The listing builds one solid part. Answer for the finished solid, in the listing's coordinates (mm). Coordinates: 2 decimals unless noted, no trailing zeros. Loops run counter-clockwise (first coordinate to the right, second up) from the corner with the lowest first, then second, coordinate; pieces in that order, holes last. Notation, with made-up numbers: M 40,71.25 L 93,71.25 A13 cw 93,95.25 Z; hole C 7,-29 d3. An arc over 180 degrees is marked long. Return JSON: item names as keys, results as strings. Group by question number.
1. Section A-A (z = -1.5) is taken. Write down the section's boundary in (x, y), then the cut area to 3 significant figures.
2. Section B-B (y = -175) is taken. Write down the section's boundary in (x, z).
3. Straight lines are drawn through the part: L1, parallel to Y at x = 4, z = -1.4; L2, parallel to Y at x = 3.25, z = 2.5; L3, parallel to X at y = -223.5, z = 0.25. For each, find the intervals that lie inside material, in ascending order. Write a range as from..to.
```python
from build123d import *

# Parameters (mm, degrees)
BOSS_EXTRUDE1_DEPTH = 400
CUT_EXTRUDE1_DEPTH  = 401.196201881
SKETCH3_R           = 1.75
CUT_EXTRUDE2_DEPTH  = 401.196201985


with BuildPart() as part:
    # Sketch1 → Boss-Extrude1 (new body)
    with BuildSketch(Plane(origin=(0, 0, 0), x_dir=(1, 0, 0), z_dir=(0, 1, 0))):
        with BuildLine():
            Line((0, 3), (8, 3))
            ThreePointArc((8, 3), (11, 0), (8, -3))
            Line((8, -3), (0, -3))
            ThreePointArc((0, -3), (-3, 0), (0, 3))
        make_face()
    extrude(amount=-BOSS_EXTRUDE1_DEPTH)

    # Sketch2 → Cut-Extrude1 (cut, through all)
    with BuildSketch(Plane(origin=(0, 0, -3), x_dir=(-1, 0, 0), z_dir=(0, 0, -1))):
        with BuildLine():
            Line((9.595782006, 3.055219164), (9.595782006, -10.123279697))
            Line((9.595782006, -10.123279697), (3.026265269, -10.123279697))
            ThreePointArc((3.026265269, -10.123279697), (-4, 0), (-11.026265269, -10.123279697))
            Line((-11.026265269, -10.123279697), (-18.139014199, -10.123279697))
            Line((-18.139014199, -10.123279697), (-18.139014199, 3.055219164))
            Line((-18.139014199, 3.055219164), (9.595782006, 3.055219164))
        make_face()
    extrude(amount=-CUT_EXTRUDE1_DEPTH, mode=Mode.SUBTRACT)

    # Sketch3 → Cut-Extrude2 (cut, through all)
    with BuildSketch(Plane.XY.offset(3)):
        with Locations((4, -7.883965637)):
            Circle(SKETCH3_R)
    extrude(amount=-CUT_EXTRUDE2_DEPTH, mode=Mode.SUBTRACT)


solid = part.part
```
Worked out:
{
 "1": {"outline": "M -2.6,-400 L 10.6,-400 L 10.6,-3.93 A7.5 ccw -2.6,-3.93 Z; hole C 4,-7.88 d3.5", "area": "5,250 mm^2"},
 "2": {"outline": "M 0,-3 L 8,-3 A3 ccw 8,3 L 0,3 A3 ccw Z"},
 "3": {"L1": "-400..-9.63, -6.13..0", "L2": "-400..-9.47, -6.3..-0.04", "L3": "-2.99..10.99"}
}
